```python
from build123d import *

# Parameters (mm, degrees)
EXTRUDE_1_DEPTH          = 5.75
EXTRUDE_1_DEPTH_BACK     = 5.75
CUT_EXTRUDE_1_DEPTH      = 30
EXTRUDE_2_DEPTH          = 40.1
CUT_EXTRUDE_2_DEPTH      = 20.2
CUT_EXTRUDE_3_DEPTH      = 4.25
CUT_EXTRUDE_3_DEPTH_BACK = 4.25
CUT_EXTRUDE_4_DEPTH      = 4.25
CUT_EXTRUDE_4_DEPTH_BACK = 4.25
CUT_EXTRUDE_5_DEPTH      = 4.25
CUT_EXTRUDE_5_DEPTH_BACK = 4.25
SKETCH_10_W              = 4
SKETCH_10_H              = 2


with BuildPart() as part:
    # 草图1 → 凸台-拉伸1 (new, two sides: drawn at the far end of the back side and taken through both)
    with BuildSketch(Plane.XY.offset(-EXTRUDE_1_DEPTH_BACK)):
        with BuildLine():
            Line((-30, 17), (-30, 15))
            Line((-30, 15), (-29, 15))
            Line((-29, 15), (-29, -15))
            Line((-29, -15), (-30, -15))
            Line((-30, -15), (-30, -33))
            Line((-30, -33), (-25.3, -33))
            ThreePointArc((-25.3, -33), (-25.087867966, -32.912132034), (-25, -32.7))
            Line((-25, -32.7), (-25, -19))
            Line((-25, -19), (-23, -17))
            Line((-23, -17), (0, -17))
            Line((0, -17), (0, -19.5))
            ThreePointArc((0, -19.5), (0.146446609, -19.853553391), (0.5, -20))
            Line((0.5, -20), (9.6, -20))
            ThreePointArc((9.6, -20), (9.953553391, -19.853553391), (10.1, -19.5))
            Line((10.1, -19.5), (10.1, 17))
            Line((10.1, 17), (-30, 17))
        make_face()
    extrude(amount=EXTRUDE_1_DEPTH + EXTRUDE_1_DEPTH_BACK)

    # 草图2 → 切除-拉伸1 (cut)
    with BuildSketch(Plane(origin=(0, 0, 0), x_dir=(0, 0, -1), z_dir=(1, 0, 0))):
        with BuildLine():
            Line((-2.75, -23.5), (-2.75, -26.5))
            ThreePointArc((-2.75, -26.5), (0, -29.25), (2.75, -26.5))
            Line((2.75, -26.5), (2.75, -23.5))
            ThreePointArc((2.75, -23.5), (0, -20.75), (-2.75, -23.5))
        make_face()
    extrude(amount=-CUT_EXTRUDE_1_DEPTH, mode=Mode.SUBTRACT)

    # 草图3 → 凸台-拉伸2 (add)
    with BuildSketch(Plane(origin=(10.1, 0, 0), x_dir=(0, 0, -1), z_dir=(1, 0, 0))):
        with BuildLine():
            Line((-5.75, 17), (5.75, 17))
            ThreePointArc((5.75, 17), (0, 18.299606469), (-5.75, 17))
        make_face()
    extrude(amount=-EXTRUDE_2_DEPTH)

    # 草图4 → 切除-旋转1 (revolve, cut)
    with BuildSketch(Plane.XY, mode=Mode.PRIVATE) as cut_revolve_1_sk:
        Polygon((4, -15), (4, -13), (11, -13), (11, -11.25), (14.5, -11.25), (15, -10.75), (15, -15), align=None)
    revolve(cut_revolve_1_sk.sketch.rotate(Axis((15, -15, 0), (-1, 0, 0)), 270), axis=Axis((15, -15, 0), (-1, 0, 0)), mode=Mode.SUBTRACT)

    # 草图5 → 切除-旋转2 (revolve, cut)
    with BuildSketch(Plane.XY, mode=Mode.PRIVATE) as cut_revolve_2_sk:
        Polygon((15, 13.75), (15, 9.5), (14.5, 10), (11, 10), (11, 11.75), (4, 11.75), (4, 13.75), align=None)
    revolve(cut_revolve_2_sk.sketch.rotate(Axis((4, 13.75, 0), (1, 0, 0)), 90), axis=Axis((4, 13.75, 0), (1, 0, 0)), mode=Mode.SUBTRACT)

    # 草图6 → 切除-拉伸2 (cut)
    with BuildSketch(Plane(origin=(10.1, 0, 0), x_dir=(0, 0, -1), z_dir=(1, 0, 0))):
        Polygon((-5.75, -8.5), (-4.9, -8.5), (-4.5, -10.1), (-0.85, -10.1), (-0.85, -10.5), (0.85, -10.5), (0.85, -10.1), (4.5, -10.1), (4.9, -8.5), (5.75, -8.5), (5.75, 8.5), (4.9, 8.5), (4.5, 10.1), (0.85, 10.1), (0.85, 10.5), (-0.85, 10.5), (-0.85, 10.1), (-4.5, 10.1), (-4.9, 8.5), (-5.75, 8.5), align=None)
    extrude(amount=-CUT_EXTRUDE_2_DEPTH, mode=Mode.SUBTRACT)

    # 草图7 → 旋转1 (revolve)
    with BuildSketch(Plane(origin=(0, 0, 0), x_dir=(0, 0, -1), z_dir=(1, 0, 0)), mode=Mode.PRIVATE) as revolve_1_sk:
        with BuildLine():
            Line((-0.75, 5), (0.75, 5))
            ThreePointArc((0.75, 5), (1.500003023, 7.375), (0.75, 9.75))
            Line((0.75, 9.75), (0.75, 10.25))
            Line((0.75, 10.25), (-0.75, 10.25))
            Line((-0.75, 10.25), (-0.75, 9.75))
            ThreePointArc((-0.75, 9.75), (-1.500003023, 7.375), (-0.75, 5))
        make_face()
    revolve(revolve_1_sk.sketch.rotate(Axis((0, 0, -50), (0, 0, 1)), 270), axis=Axis((0, 0, -50), (0, 0, 1)))

    # 草图8 → 切除-拉伸3 (cut, two sides: drawn at the far end of the back side and taken through both)
    with BuildSketch(Plane.XY.offset(-CUT_EXTRUDE_3_DEPTH_BACK)):
        Polygon((-29, 13.535533906), (-29, 1), (-13.535533906, 1), (-13.535533906, 8.535533906), (-8.535533906, 13.535533906), align=None)
    extrude(amount=CUT_EXTRUDE_3_DEPTH + CUT_EXTRUDE_3_DEPTH_BACK, mode=Mode.SUBTRACT)

    # 草图9 → 切除-拉伸4 (cut, two sides: drawn at the far end of the back side and taken through both)
    with BuildSketch(Plane.XY.offset(-CUT_EXTRUDE_4_DEPTH_BACK)):
        Polygon((-29, -13.535533906), (-8.535533906, -13.535533906), (-13.535533906, -8.535533906), (-13.535533906, -1), (-29, -1), align=None)
    extrude(amount=CUT_EXTRUDE_4_DEPTH + CUT_EXTRUDE_4_DEPTH_BACK, mode=Mode.SUBTRACT)

    # 草图10 → 切除-拉伸5 (cut, two sides: drawn at the far end of the back side and taken through both)
    with BuildSketch(Plane.XY.offset(-CUT_EXTRUDE_5_DEPTH_BACK)):
        with Locations((-27, 0)):
            Rectangle(SKETCH_10_W, SKETCH_10_H)
    extrude(amount=CUT_EXTRUDE_5_DEPTH + CUT_EXTRUDE_5_DEPTH_BACK, mode=Mode.SUBTRACT)


solid = part.part
```
The model under review builds one solid part; all positions refer to its coordinate system, in mm. A direction names the side the tool comes from. Give positions to 0.01 mm unless a question says otherwise; leave off trailing zeros. Write each loop counter-clockwise with the first axis right and the second up, starting at its lowest first coordinate (ties: lowest second). Pieces come first, ordered by that corner, then holes.
(1) To check wall thickness, follow L1, parallel to X at y = -19.5, z = 4.75; L2, parallel to Z at x = -16, y = 11.5; L3, parallel to Z at x = 6, y = -15. State the ranges of each line that lie inside material, in increasing order.
(2) Tool access review of faces 4 (the flat face through (3.9, -9.1, -0.75)), 5 (the flat face through (-29.5, -15, -0.1)), 6 (the flat face through (-27, -25, 2.75)), 7 (the flat face through (-25, -27, -3)), 8 (the flat face through (-21, 3, 4.25)): name each direction out of +Z, -Z, +X, -X, +Y, -Y from which nothing blocks a thin tool from reaching the whole face with its end or side.
(3) Consider section A-A, the plane y = 0. Give the boundary of the cut face in (x, z) (3 decimals), and give its area (3 significant figures).
(4) The part is to be moulded in two halves that separate along Z. For faces 1 (the flat face through (-30, 16, 0)), 2 (the flat face through (-15, -2, -5.75)), 3 (the flat face through (0, 10.1, 3)), say which applies: released by +Z, released by -Z, zero draft, split by the parting line, or undercut.
(5) Consider section B-B, the plane z = 0. Give the number of separate pieces and of enclosed holes in the cut face, and give its area (3 significant figures).
(6) Consider section C-C, the plane y = -12. Give the boundary of the cut face in (x, z).
(7) For P1, Ø1, axis at y = 4, z = 3.5, coming from the +X side; P2, Ø3.5, axis at y = -28, z = -1.5, coming from the +X side; P3, Ø3, axis at y = -19, z = 0, coming from the +X side, all flat-tipped, find the tip position at first contact; note any pin that passes through.
Returned:
1. L1: x = -30 to -25, 0 to 10.1
1. L2: z = -5.75 to -4.25, 4.25 to 5.75
1. L3: z = -5.75 to -2, 2 to 5.75
2. face 4: none
2. face 5: +Z, -Z, -X
2. face 6: +X, -X
2. face 7: +Z, -Z, -Y
2. face 8: -X
3. outline: (-29, -5.75) - (-10.1, -5.75) - (-10.1, -0.75) - (-9.75, -0.75) arc R4.135 ccw to (-5, -0.75) - (-5, 0.75) arc R4.135 ccw to (-9.75, 0.75) - (-10.1, 0.75) - (-10.1, 5.75) - (-29, 5.75) - (-29, 4.25) - (-25, 4.25) - (-25, -4.25) - (-29, -4.25) - close; (5, -0.75) arc R4.135 ccw to (9.75, -0.75) - (10.25, -0.75) - (10.25, 0.75) - (9.75, 0.75) arc R4.135 ccw to (5, 0.75) - close
3. area: 209 mm2
4. face 1: zero draft
4. face 2: released by -Z
4. face 3: undercut
5. separate pieces: 2
5. enclosed holes: 1
5. area: 813 mm2
6. outline: (-29, -5.75) - (10.1, -5.75) - (10.1, 5.75) - (-29, 5.75) - (-29, 4.25) - (-10.07, 4.25) - (-10.07, -4.25) - (-29, -4.25) - close
7. P1: stops at x = -10.1
7. P2: stops at x = -25
7. P3: stops at x = 10.1
